```python
from build123d import *

# Parameters (mm, degrees)
SKETCH_1_W               = 179
SKETCH_1_H               = 15
FILLET_1_R               = 0.5
EXTRUDE_START            = 13
SKETCH_2_R               = 58
SKETCH_2_R_2             = 25
EXTRUDE_1_DEPTH          = 13
SKETCH_3_W               = 8.1
SKETCH_3_H               = 7
SKETCH_3_W_2             = 4.9
SKETCH_3_H_2             = 4.5
PATTERN_CIRCULAR_1_COUNT = 4


with BuildPart() as part:
    # 草图1 → 旋转1 (revolve)
    with BuildSketch(Plane(origin=(0, 0, 0), x_dir=(0, 0, -1), z_dir=(1, 0, 0)), mode=Mode.PRIVATE) as revolve_1_sk:
        with Locations((89.5, 32.5)):
            Rectangle(SKETCH_1_W, SKETCH_1_H)
    revolve(revolve_1_sk.sketch.rotate(Axis((0, 0, 0), (0, 0, -1)), 90), axis=Axis((0, 0, 0), (0, 0, -1)))

    # 圆角1
    fillet_1_edges = [part.edges().sort_by_distance(p)[0] for p in [
        (-40, 0, -179),
    ]]
    fillet(fillet_1_edges, radius=FILLET_1_R)

    # 草图2 → 凸台-拉伸1 (add)
    with BuildSketch(Plane.XY.offset(EXTRUDE_START)):
        with Locations(Location((0, 0, 0), (0, 0, 180))):
            Circle(SKETCH_2_R)
        Circle(SKETCH_2_R_2, mode=Mode.SUBTRACT)
    extrude(amount=-EXTRUDE_1_DEPTH)

    # 草图3 → 切除-旋转1 (revolve, cut)
    with BuildSketch(Plane(origin=(0, 0, 0), x_dir=(0, 0, -1), z_dir=(1, 0, 0)), mode=Mode.PRIVATE) as cut_revolve_1_sk:
        with Locations((-8.95, 52.5)):
            Rectangle(SKETCH_3_W, SKETCH_3_H)
        Polygon((-4.9, 56), (-13, 56), (-13, 49), (-4.9, 49), (-4.9, 53.5), align=None)
        with Locations((-2.45, 51.25)):
            Rectangle(SKETCH_3_W_2, SKETCH_3_H_2)
    cut_revolve_1 = revolve(cut_revolve_1_sk.sketch.rotate(Axis((0, 49, 0), (0, 0, -1)), 90), axis=Axis((0, 49, 0), (0, 0, -1)), mode=Mode.SUBTRACT)

    # 阵列(圆周)1: 切除-旋转1 ×4 about axis
    pattern_circular_1_axis = Axis((0, 0, 0), (0, 0, 1))
    for i in range(1, PATTERN_CIRCULAR_1_COUNT):
        add(cut_revolve_1.rotate(pattern_circular_1_axis, i * 360 / PATTERN_CIRCULAR_1_COUNT), mode=Mode.SUBTRACT)


solid = part.part
```
Here's how the part is built. I have some questions about the finished solid (model axes, mm). A direction names the side the tool comes from. Give positions to 0.01 mm unless a question says otherwise; leave off trailing zeros. Write each loop counter-clockwise with the first axis right and the second up, starting at its lowest first coordinate (ties: lowest second). Pieces come first, ordered by that corner, then holes. Notation, with made-up numbers: (87, 72) -> (136, 72) arc R10 ccw to (136, 88) -> close; hole circle Ø3 at (81, 67.25). An arc over 180 degrees is marked (long way). Use one line per item in the form item = value.
1) Suppose I cut it at A-A (x = 0). Give the number of separate pieces and of enclosed holes in the cut face, and give its area (3 significant figures).
Verdict:
separate_pieces = 4
enclosed_holes = 0
area = 5,910 mm2
2) I'm going to push flat-ended pins straight in: pin 1 (11.5 mm diameter, centred on x = 49, y = 0, fed in from -Z); pin 2 (8 mm diameter, centred on y = -15, z = -123.5, fed in from +X); pin 3 (11.5 mm diameter, centred on x = -49, y = 0, fed in from +Z); pin 4 (18 mm diameter, centred on x = 0, y = -49, fed in from +Z). Where does each tip first touch, or does it pass through?
Verdict:
pin_1 = 0
pin_2 = 38.46
pin_3 = 4.9
pin_4 = 13
3) Suppose I cut it at C-C (y = -49). Please give me the cut outline in (x, z).
Verdict:
outline = (-31.03, 0) -> (-4.5, 0) -> (-4.5, 4.9) -> (-7, 4.9) -> (-7, 13) -> (-31.03, 13) -> close; (4.5, 0) -> (31.03, 0) -> (31.03, 13) -> (7, 13) -> (7, 4.9) -> (4.5, 4.9) -> close
4) On a 3-axis mill with a long thin cutter (end or side, diameter ignored), from which of +Z, -Z, +X, -X, +Y, -Y can I reach the whole of each face in a straight line? I mean faces 1 (the face through (-39.96, -1.76, -90.5)), 2 (the face through (23.846, 7.509, -81.656)), 3 (the face through (49, 5, 4.9)). Say none if no direction works.
Verdict:
face_1 = -Z
face_2 = +Z, -Z
face_3 = +Z
5) We'd pull the mould along Y, two halves only. Please class faces 4 (the face through (14, 38, 0)), 5 (the face through (-26.76, 51.46, 6.59)), 6 (the face through (0.91, -42.06, 8.89)): +Y half, -Y half, draft (parallel to the pull), parting line (faces both ways), or undercut.
Verdict:
face_4 = draft
face_5 = parting line
face_6 = undercut
6) If I drill on L1, parallel to Y at x = 18, z = -127; L2, parallel to Z at x = 53.5, y = 11; L3, parallel to Z at x = 50, y = -6, over which ranges is the centre line in solid material (lowest first)? Write a range as [from, to].
Verdict:
L1 = [-35.72, -17.35], [17.35, 35.72]
L2 = [0, 13]
L3 = [0, 4.9]
